Design review of the part built by this model. Coordinates are the model's own, in mm. A direction names the side the tool comes from. Coordinates: 2 decimals unless noted, no trailing zeros. Write each loop counter-clockwise with the first axis right and the second up, starting at its lowest first coordinate (ties: lowest second). Pieces come first, ordered by that corner, then holes.
```python
from build123d import *

# Parameters (mm, degrees)
SKETCH_1_W          = 180
SKETCH_1_H          = 150
EXTRUDE_1_DEPTH     = 10
CUT_EXTRUDE_1_REACH = 119.58
SKETCH_2_W          = 20
SKETCH_2_H          = 100


with BuildPart() as part:
    # 草图1 → 凸台-拉伸1 (new body)
    with BuildSketch(Plane.XY):
        Rectangle(SKETCH_1_W, SKETCH_1_H)
    extrude(amount=EXTRUDE_1_DEPTH)

    # 草图2 → 切除-拉伸1 (cut, up to next)
    with BuildSketch(Plane.XY.offset(10), mode=Mode.PRIVATE) as cut_extrude_1_sk1:
        with Locations((-45, -25)):
            Rectangle(SKETCH_2_W, SKETCH_2_H)
    cut_extrude_1_tool1 = extrude(cut_extrude_1_sk1.sketch, amount=-CUT_EXTRUDE_1_REACH, mode=Mode.PRIVATE) & part.part
    cut_extrude_1 = cut_extrude_1_tool1.solids().sort_by_distance((-45, -25, 10))[0]
    add(cut_extrude_1, mode=Mode.SUBTRACT)

    # 镜向1: 切除-拉伸1 across plane
    add(cut_extrude_1.mirror(Plane(origin=(0, 0, 0), x_dir=(0, 0, 1), z_dir=(1, 0, 0))), mode=Mode.SUBTRACT)


solid = part.part
```
(1) Consider section A-A (y = 12). Give the boundary of the cut face in (x, z), plus the area to 3 significant figures.
(2) Consider section B-B (z = 4.5). Give the boundary of the cut face in (x, y).
(3) For faces 4 (the flat face through (55, -26, 5)), 5 (the flat face through (-1, 1, 10)), list the 3-axis set-ups (+Z, -Z, +X, -X, +Y, -Y) from which the entire face can be reached by the end or side of a thin tool; tool diameter is ignored.
(4) Mouldability with a two-part tool opening along X and no side actions: class faces 1 (the flat face through (-90, -1, 5)), 2 (the flat face through (0, -75, 5)), 3 (the flat face through (-55, -26, 5)) as +X half, -X half, draft (parallel to the pull), parting line (faces both ways), or undercut.
(5) Wall thickness on line 1 (X direction, y = 1, z = 2.25); line 2 (Y direction, x = 46, z = 9): over which ranges is each line inside the solid? List them lowest first.
(6) Consider section C-C (x = -52). Give the boundary of the cut face in (y, z), plus the area to 3 significant figures.
(7) Insertion check: pin 1 Ø5 at (x, z) = (45.5, 6.5) entering from -Y. The pin has a flat end and moves straight along its axis. Give the tip position at first contact, or say it passes through.
Results:
1. outline: (-90, 0) - (-55, 0) - (-55, 10) - (-90, 10) - close; (-35, 0) - (35, 0) - (35, 10) - (-35, 10) - close; (55, 0) - (90, 0) - (90, 10) - (55, 10) - close
1. area: 1,400 mm2
2. outline: (-90, -75) - (-55, -75) - (-55, 25) - (-35, 25) - (-35, -75) - (35, -75) - (35, 25) - (55, 25) - (55, -75) - (90, -75) - (90, 75) - (-90, 75) - close
3. face 4: +Z, -Z, -Y
3. face 5: +Z, +X, -X, +Y, -Y
4. face 1: -X half
4. face 2: draft
4. face 3: undercut
5. line 1: x = -90 to -55, -35 to 35, 55 to 90
5. line 2: y = 25 to 75
6. outline: (25, 0) - (75, 0) - (75, 10) - (25, 10) - close
6. area: 500 mm2
7. pin 1: stops at y = 25
